Design review of the part built by this model. Coordinates are the model's own, in mm. Face numbers are marked on the shaded views. A direction names the side the tool comes from. Give positions to 0.01 mm unless a question says otherwise; leave off trailing zeros. Order: outer loops, then holes, each group sorted by start corner. A loop starts at its lowest first (then second) coordinate and runs counter-clockwise, first axis right, second up. Notation, with made-up numbers: (69, 17.25) - (109, 17.25) arc R24 cw to (109, 54.25) - close; hole circle Ø5 at (87.5, 33.5). An arc over 180 degrees is marked (long way). Write each question's results on one line, items separated by ' | '. Start each with the question number.
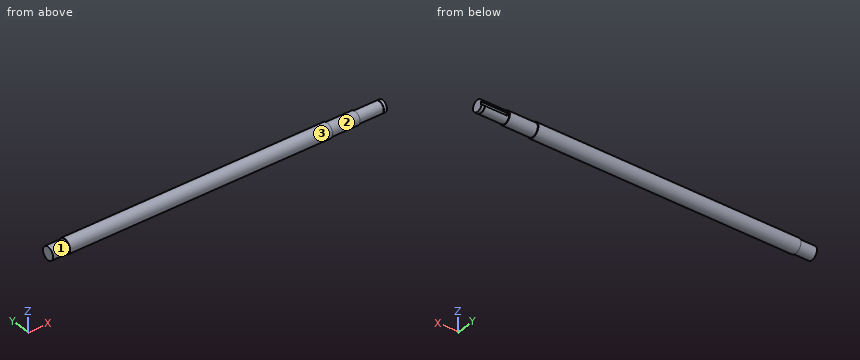
```python
from build123d import *

# Parameters (mm, degrees)
CUT_EXTRUDE_1_DEPTH = 5
SKETCH_3_R          = 20
SKETCH_3_R_2        = 18.75
CUT_EXTRUDE_2_DEPTH = 1.7


with BuildPart() as part:
    # 草图1 → 旋转1 (revolve)
    with BuildSketch(Plane.XY):
        Polygon((0, 0), (0, 22.5), (58, 22.5), (58, 25), (978, 25), (978, 22.5), (1076, 22.5), (1076, 20), (1172, 20), (1172, 0), align=None)
    revolve(axis=Axis((1172, 0, 0), (-1, 0, 0)))

    # 草图2 → 切除-拉伸1 (cut)
    with BuildSketch(Plane(origin=(0, 20, 0), x_dir=(1, 0, 0), z_dir=(0, 1, 0))):
        with BuildLine():
            Line((1086, 6), (1182, 6))
            Line((1182, 6), (1182, -6))
            Line((1182, -6), (1086, -6))
            ThreePointArc((1086, -6), (1080, 0), (1086, 6))
        make_face()
    extrude(amount=-CUT_EXTRUDE_1_DEPTH, mode=Mode.SUBTRACT)

    # 草图3 → 切除-拉伸2 (cut)
    with BuildSketch(Plane(origin=(1161.5, 0, 0), x_dir=(0, 0, -1), z_dir=(1, 0, 0))):
        with Locations(Location((0, 0, 0), (0, 0, 90))):
            Circle(SKETCH_3_R)
        Circle(SKETCH_3_R_2, mode=Mode.SUBTRACT)
    extrude(amount=-CUT_EXTRUDE_2_DEPTH, mode=Mode.SUBTRACT)


solid = part.part
```
Q1. For line 1 (X direction, y = 18, z = 8.5); line 2 (Z direction, x = 782, y = 15); line 3 (Y direction, x = 310, z = 2), list the stretches that pass through material, from the lowest coordinate up. Write a range as [from, to].
Q2. Add section B-B (x = 673.5). Give the boundary of the cut face in (y, z), plus the area to 3 significant figures.
Q3. Insertion check: pin 1 Ø1.5 at (x, z) = (380.5, -5.5) entering from -Y; pin 2 Ø10 at (x, y) = (502, -18.5) entering from +Z; pin 3 Ø1 at (x, y) = (1048, 2) entering from +Z. Each pin has a flat end and moves straight along its axis. Give the tip position at first contact, or say it passes through.
Q4. Add section A-A (y = 0). Give the boundary of the cut face in (x, z).
Q5. Machinability: for the marked faces 1, 2 and 3, which of the approach directions +Z, -Z, +X, -X, +Y, -Y give a long, thin tool a straight path to every point of the face, cutting with its end or side? Answer none if there is none.
Verdict:
1) line 1: x = [0, 1159.8], [1161.5, 1172] | line 2: z = [-20, 20] | line 3: y = [-24.92, 24.92]
2) outline: circle Ø50 at (0, 0) | area: 1,960 mm2
3) pin 1: stops at y = -24.54 | pin 2: stops at z = 21.04 | pin 3: stops at z = 22.45
4) outline: (0, -22.5) - (58, -22.5) - (58, -25) - (978, -25) - (978, -22.5) - (1076, -22.5) - (1076, -20) - (1159.8, -20) - (1159.8, -18.75) - (1161.5, -18.75) - (1161.5, -20) - (1172, -20) - (1172, 20) - (1161.5, 20) - (1161.5, 18.75) - (1159.8, 18.75) - (1159.8, 20) - (1076, 20) - (1076, 22.5) - (978, 22.5) - (978, 25) - (58, 25) - (58, 22.5) - (0, 22.5) - close
5) face 1: -X | face 2: +X | face 3: +X, -X
